```python
from build123d import *

# Parameters (mm, degrees)
SKETCH_1_R      = 2.25
EXTRUDE_1_DEPTH = 21
EXTRUDE_3_DEPTH = 21


with BuildPart() as part:
    # 草图1 → 凸台-拉伸1 (new body)
    with BuildSketch(Plane.XY):
        Polygon((0, 0), (70, 0), (70, 20), (54, 20), (54, 37), (0, 37), align=None)
        with Locations(Location((14, 18, 0), (0, 0, 180))):
            Circle(SKETCH_1_R, mode=Mode.SUBTRACT)
        with Locations(Location((40, 18, 0), (0, 0, 180))):
            Circle(SKETCH_1_R, mode=Mode.SUBTRACT)
    extrude(amount=EXTRUDE_1_DEPTH)

    # 草图2 → 凸台-拉伸3 (add)
    with BuildSketch(Plane.XY.offset(21)):
        with BuildLine():
            Line((62.423710356, 40.295115228), (74.506235043, 32.160250075))
            Line((74.506235043, 32.160250075), (73.947745443, 31.330738552))
            Line((73.947745443, 31.330738552), (62.118443298, 39.295115228))
            ThreePointArc((62.118443298, 39.295115228), (59.453208897, 40.564286494), (56.533547297, 41))
            Line((56.533547297, 41), (1, 41))
            Line((1, 41), (1, 37))
            Line((1, 37), (0, 37))
            Line((0, 37), (0, 42))
            Line((0, 42), (56.838814355, 42))
            ThreePointArc((56.838814355, 42), (59.758475955, 41.564286494), (62.423710356, 40.295115228))
        make_face()
    extrude(amount=-EXTRUDE_3_DEPTH)


solid = part.part
```
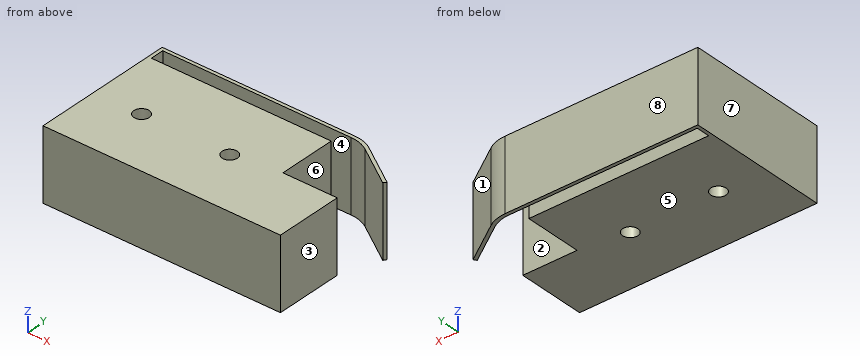
Input: part model. Units: mm. Frame: model coordinates. Face numbers are marked on the shaded views. A direction names the side the tool comes from. Round coordinates to 2 decimals unless told otherwise and drop trailing zeros. Loops run counter-clockwise (first coordinate to the right, second up) from the corner with the lowest first, then second, coordinate; pieces in that order, holes last. Notation, with made-up numbers: (87, 83) -> (125, 83) arc R35 cw to (125, 116) -> close; hole circle Ø2 at (80, 15). An arc over 180 degrees is marked (long way). One line per item, written item: value.
(1) Section C-C (y = 18). Return the cut outline in (x, z).
Geometry check:
outline: (0, 0) -> (11.75, 0) -> (11.75, 21) -> (0, 21) -> close; (16.25, 0) -> (37.75, 0) -> (37.75, 21) -> (16.25, 21) -> close; (42.25, 0) -> (70, 0) -> (70, 21) -> (42.25, 21) -> close
(2) Material intervals for line 1 (X direction, y = 18, z = 13.5); line 2 (Y direction, x = 14, z = 13); line 3 (Y direction, x = 29, z = 10.5), sorted ascending. Write a range as [from, to].
Geometry check:
line 1: [0, 11.75], [16.25, 37.75], [42.25, 70]
line 2: [0, 15.75], [20.25, 37], [41, 42]
line 3: [0, 37], [41, 42]
(3) Set-up query: the marked faces 1, 2, 3, 4 and 5. Return all of +Z, -Z, +X, -X, +Y, -Y with unobstructed straight access to the full face (end or side cutting, diameter ignored); none if empty.
Geometry check:
face 1: +Z, -Z, +X, +Y
face 2: +Z, -Z, +X
face 3: +Z, -Z, +X, -Y
face 4: +Z, -Z
face 5: -Z, +X, -X, +Y, -Y
(4) Mould query, pull axis X, two halves, no side actions, for the marked faces 6, 7 and 8. Classes: pulls with the +X half, pulls with the -X half, needs draft (parallel to the pull), parting line crosses it, or undercut.
Geometry check:
face 6: undercut
face 7: pulls with the -X half
face 8: needs draft
(5) Section A-A (x = 40). Return the cut outline in (y, z), plus the area to 4 significant figures.
Geometry check:
outline: (0, 0) -> (15.75, 0) -> (15.75, 21) -> (0, 21) -> close; (20.25, 0) -> (37, 0) -> (37, 21) -> (20.25, 21) -> close; (41, 0) -> (42, 0) -> (42, 21) -> (41, 21) -> close
area: 703.5 mm2
(6) Section B-B (z = 14). Return the cut outline in (x, y).
Geometry check:
outline: (0, 0) -> (70, 0) -> (70, 20) -> (54, 20) -> (54, 37) -> (1, 37) -> (1, 41) -> (56.53, 41) arc R10 cw to (62.12, 39.3) -> (73.95, 31.33) -> (74.51, 32.16) -> (62.42, 40.3) arc R10 ccw to (56.84, 42) -> (0, 42) -> close; hole circle Ø4.5 at (14, 18); hole circle Ø4.5 at (40, 18)
(7) Section D-D (x = 49.5). Return the cut outline in (y, z).
Geometry check:
outline: (0, 0) -> (37, 0) -> (37, 21) -> (0, 21) -> close; (41, 0) -> (42, 0) -> (42, 21) -> (41, 21) -> close
(8) Pin query (flat end, axial travel): pin 1 (1.2 mm diameter, centred on y = 40, z = 8, fed in from +X); pin 2 (10 mm diameter, centred on y = 9, z = 6, fed in from +X); pin 3 (5 mm diameter, centred on y = 27, z = 7.5, fed in from +X). Return the tip coordinate at first contact, or that it passes through.
Geometry check:
pin 1: x = 63.75
pin 2: x = 70
pin 3: x = 54
